from build123d import *

# Parameters (mm, degrees)
SKETCH1_W           = 77
SKETCH1_H           = 238
BOSS_EXTRUDE1_DEPTH = 1
SKETCH2_W           = 77
SKETCH2_H           = 1
BOSS_EXTRUDE2_DEPTH = 38
BOSS_EXTRUDE3_DEPTH = 1


with BuildPart() as part:
    # Sketch1 → Boss-Extrude1 (new body)
    with BuildSketch(Plane.XY):
        Rectangle(SKETCH1_W, SKETCH1_H)
    extrude(amount=BOSS_EXTRUDE1_DEPTH)

    # Sketch2 → Boss-Extrude2 (add)
    with BuildSketch(Plane.XY.offset(1)):
        with Locations((0, 118.5)):
            Rectangle(SKETCH2_W, SKETCH2_H)
        with Locations((0, -118.5)):
            Rectangle(SKETCH2_W, SKETCH2_H)
    extrude(amount=BOSS_EXTRUDE2_DEPTH)

    # Sketch3 → Boss-Extrude3 (add)
    with BuildSketch(Plane.ZY.offset(38.5)):
        Polygon((2, 119), (0, 119), (0, -119), (39, -119), (39, -118), (1, -118), (1, 118), (2, 118), align=None)
    extrude(amount=BOSS_EXTRUDE3_DEPTH)


solid = part.part
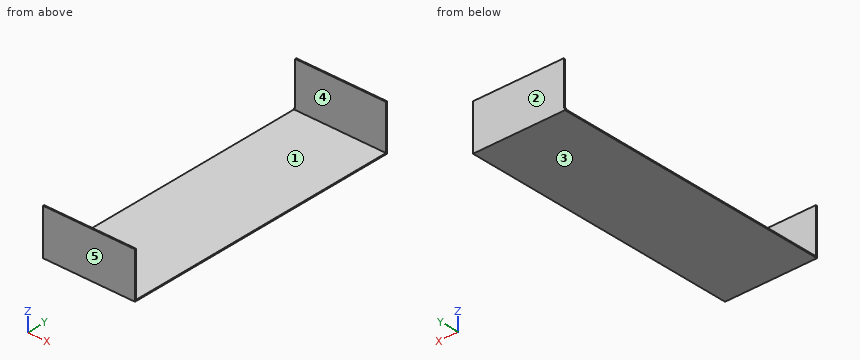
Part model, mm, in its own coordinate system. Face numbers are marked on the shaded views. A direction names the side the tool comes from. Give positions to 0.01 mm unless a question says otherwise; leave off trailing zeros. Write each loop counter-clockwise with the first axis right and the second up, starting at its lowest first coordinate (ties: lowest second). Pieces come first, ordered by that corner, then holes.
1) Which spindle directions (+Z, -Z, +X, -X, +Y, -Y) get a long thin tool onto all of the face, cutting with end or side? Do the marked faces 4 and 5. Say none if no direction does.
Resolved:
face 4: +Z, +X, -X
face 5: +Z, -Z, +X, -X, -Y
2) Two-plate mould, pull along Y, no slides. Class the marked faces 1, 2 and 3: released by +Y, released by -Y, zero draft, split by the parting line, or undercut.
Resolved:
face 1: undercut
face 2: released by +Y
face 3: zero draft
3) Cut at B-B on x = 5.5. Write the cut outline in (y, z), then the cut area to 3 significant figures.
Resolved:
outline: (-119, 0) - (119, 0) - (119, 39) - (118, 39) - (118, 1) - (-118, 1) - (-118, 39) - (-119, 39) - close
area: 314 mm2
4) Cut at C-C on y = 45. Write the cut outline in (x, z).
Resolved:
outline: (-39.5, 0) - (38.5, 0) - (38.5, 1) - (-39.5, 1) - close
5) Cut at A-A on z = 35. Write the cut outline in (x, y), then the cut area to 3 significant figures.
Resolved:
outline: (-39.5, -119) - (38.5, -119) - (38.5, -118) - (-39.5, -118) - close; (-38.5, 118) - (38.5, 118) - (38.5, 119) - (-38.5, 119) - close
area: 155 mm2
6) Pin check, flat tip, straight feed: pin 1 (6 mm diameter, centred on x = -26.5, y = 17, fed in from +Z). Stop position of the tip, or through.
Resolved:
pin 1: stops at z = 1
7) Probe L1, parallel to Y at x = -27, z = 13; L2, parallel to Z at x = 9, y = -71. List the from-to ranges inside material, lowest first.
Resolved:
L1: y = -119 to -118, 118 to 119
L2: z = 0 to 1
